The listing builds one solid part. Answer for the finished solid, in the listing's coordinates (mm). Round coordinates to 2 decimals unless told otherwise and drop trailing zeros. Order: outer loops, then holes, each group sorted by start corner. A loop starts at its lowest first (then second) coordinate and runs counter-clockwise, first axis right, second up. Notation, with made-up numbers: (-4.5, 78.25) -> (48.5, 78.25) arc R37 cw to (48.5, 116.25) -> close; hole circle Ø5 at (66.25, -3). An arc over 180 degrees is marked (long way). Answer in a Markdown table with one row per item. Add a question column.
```python
from build123d import *

# Parameters (mm, degrees)
SKETCH1_W           = 60
SKETCH1_H           = 40
BOSS_EXTRUDE1_DEPTH = 6
SKETCH2_R           = 4.5
CUT_EXTRUDE1_DEPTH  = 6


with BuildPart() as part:
    # Sketch1 → Boss-Extrude1 (new body)
    with BuildSketch(Plane.XY):
        Rectangle(SKETCH1_W, SKETCH1_H)
    extrude(amount=BOSS_EXTRUDE1_DEPTH)

    # Sketch2 → Cut-Extrude1 (cut)
    with BuildSketch(Plane.XY.offset(6)):
        with Locations((20.134545778, 0)):
            Circle(SKETCH2_R)
    extrude(amount=-CUT_EXTRUDE1_DEPTH, mode=Mode.SUBTRACT)


solid = part.part
```
Item 1: For a pull along X with two mould halves and no side action, classify faces 1 (the face through (-30, 0, 3)), 2 (the face through (0, -20, 3)), 3 (the face through (15.64, 0.2, 3.04)) as released by +X, released by -X, zero draft, split by the parting line, or undercut.
Item 2: The part is cut by section C-C, the plane z = 3.1. Give the vertices of the cut face in (x, y).
Item 3: Find the intervals of material crossed by probe 1 along Y at (x, z) = (19, 1.35); probe 2 along X at (y, z) = (4, 1.05); probe 3 along X at (y, z) = (3, 5.65), in increasing order. Write a range as [from, to].
Item 4: The part is cut by section A-A, the plane y = 0. Give the vertices of the cut face in (x, z).
Item 5: The part is cut by section B-B, the plane x = 17.5. Give the vertices of the cut face in (y, z), and give its area (3 significant figures).
Resolved:
| question | item | result |
|---|---|---|
| 1 | face 1 | released by -X |
| 1 | face 2 | zero draft |
| 1 | face 3 | undercut |
| 2 | outline | (-30, -20) -> (30, -20) -> (30, 20) -> (-30, 20) -> close; hole circle Ø9 at (20.13, 0) |
| 3 | probe 1 | [-20, -4.35], [4.35, 20] |
| 3 | probe 2 | [-30, 18.07], [22.2, 30] |
| 3 | probe 3 | [-30, 16.78], [23.49, 30] |
| 4 | outline | (-30, 0) -> (15.63, 0) -> (15.63, 6) -> (-30, 6) -> close; (24.63, 0) -> (30, 0) -> (30, 6) -> (24.63, 6) -> close |
| 5 | outline | (-20, 0) -> (-3.65, 0) -> (-3.65, 6) -> (-20, 6) -> close; (3.65, 0) -> (20, 0) -> (20, 6) -> (3.65, 6) -> close |
| 5 | area | 196 mm2 |
